Check sheet for the modelled part. Datum: model origin and axes. Units: mm. A direction names the side the tool comes from. Round coordinates to 2 decimals unless told otherwise and drop trailing zeros. Order: outer loops, then holes, each group sorted by start corner. A loop starts at its lowest first (then second) coordinate and runs counter-clockwise, first axis right, second up.
```python
from build123d import *

# Parameters (mm, degrees)
BOSS_EXTRUDE1_DEPTH = 480


with BuildPart() as part:
    # Sketch1 → Boss-Extrude1 (new body)
    with BuildSketch(Plane.XY):
        with BuildLine():
            Line((0, 0), (0, 19))
            Line((0, 19), (1.5, 19))
            Line((1.5, 19), (1.5, 18.5))
            Line((1.5, 18.5), (0.5, 18.5))
            Line((0.5, 18.5), (0.5, 17.5))
            Line((0.5, 17.5), (1.5, 17.5))
            ThreePointArc((1.5, 17.5), (12.813708499, 12.813708499), (17.5, 1.5))
            Line((17.5, 1.5), (17.5, 0.5))
            Line((17.5, 0.5), (18.5, 0.5))
            Line((18.5, 0.5), (18.5, 1.5))
            Line((18.5, 1.5), (19, 1.5))
            Line((19, 1.5), (19, 0))
            Line((19, 0), (16.5, 0))
            Line((16.5, 0), (16.5, 1.5))
            ThreePointArc((16.5, 1.5), (12.106601718, 12.106601718), (1.5, 16.5))
            Line((1.5, 16.5), (1.5, 0))
            Line((1.5, 0), (0, 0))
        make_face()
    extrude(amount=BOSS_EXTRUDE1_DEPTH)


solid = part.part
```
Item 1: Sectioned sample at C-C (x = 8.75). Record the cut outline in (y, z).
Answer:
outline: (14.63, 0) - (15.76, 0) - (15.76, 480) - (14.63, 480) - close
Item 2: Scan lines: line 1 along X through (y, z) = (1.25, 329); line 2 along Y through (x, z) = (1, 39.5); line 3 along Y through (x, z) = (2.75, 72.5). Record each from-to range of solid material in increasing order.
Answer:
line 1: x = 0 to 1.5, 16.5 to 17.5, 18.5 to 19
line 2: y = 0 to 17.5, 18.5 to 19
line 3: y = 16.45 to 17.45
Item 3: Release check for a two-part mould opening along X. For faces 1 (the flat face through (0, 9, 237)), 2 (the cylindrical face through (12.22, 11.99, 236.64)), 3 (the flat face through (9.5, 14.5, 480)) record: released by +X, released by -X, zero draft, split by the parting line, or undercut.
Answer:
face 1: released by -X
face 2: undercut
face 3: zero draft
Item 4: Go/stop test with flat-tipped pins: P1, Ø2, axis at x = 5, z = 422.5, coming from the -Y side; P2, Ø3, axis at x = 7.5, z = 194, coming from the +Y side; P3, Ø0.5, axis at y = 18, z = 257, coming from the +X side. Record where each tip stops, or that it passes through.
Answer:
P1: stops at y = 15.81
P2: stops at y = 16.85
P3: stops at x = 0.5
Item 5: Sectioned sample at A-A (y = 5.75). Record the cut outline in (x, z).
Answer:
outline: (0, 0) - (1.5, 0) - (1.5, 480) - (0, 480) - close; (15.89, 0) - (16.93, 0) - (16.93, 480) - (15.89, 480) - close
Item 6: Sectioned sample at B-B (z = 210). Record the cut outline in (x, y), and give its area (3 significant figures).
Answer:
outline: (0, 0) - (1.5, 0) - (1.5, 16.5) arc R15 cw to (16.5, 1.5) - (16.5, 0) - (19, 0) - (19, 1.5) - (18.5, 1.5) - (18.5, 0.5) - (17.5, 0.5) - (17.5, 1.5) arc R16 ccw to (1.5, 17.5) - (0.5, 17.5) - (0.5, 18.5) - (1.5, 18.5) - (1.5, 19) - (0, 19) - close
area: 54.6 mm2
Item 7: Access from +Z, -Z, +X, -X, +Y, -Y to the whole of each face (thin tool, end or side, straight path). Record for faces 4 (the flat face through (9.5, 14.5, 0)), 5 (the flat face through (1.5, 8, 237)).
Answer:
face 4: -Z, +X, -X, +Y, -Y
face 5: +Z, -Z, -Y
